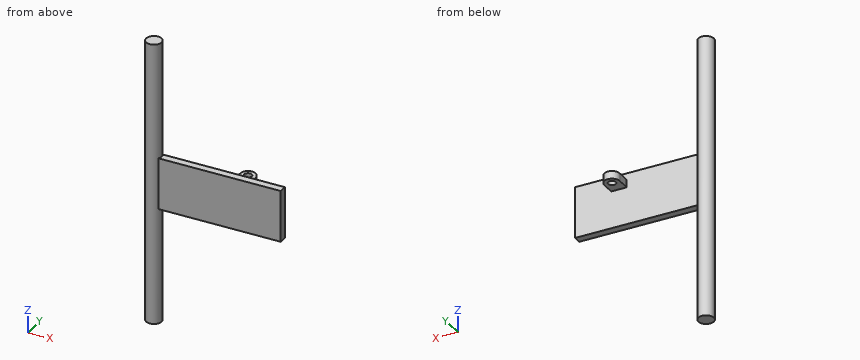
```python
from build123d import *

# Parameters (mm, degrees)
SKETCH1_R           = 3
BOSS_EXTRUDE1_DEPTH = 55
SKETCH2_W           = 50
SKETCH2_H           = 3
BOSS_EXTRUDE2_DEPTH = 10
SKETCH3_R           = 3
SKETCH3_R_2         = 1.5
BOSS_EXTRUDE3_DEPTH = 3


with BuildPart() as part:
    # Sketch1 → Boss-Extrude1 (new, symmetric)
    with BuildSketch(Plane.XY):
        Circle(SKETCH1_R)
    extrude(amount=BOSS_EXTRUDE1_DEPTH, both=True)

    # Sketch2 → Boss-Extrude2 (add, symmetric)
    with BuildSketch(Plane.XY):
        with Locations((25, 0)):
            Rectangle(SKETCH2_W, SKETCH2_H)
    extrude(amount=BOSS_EXTRUDE2_DEPTH, both=True)

    # Sketch3 → Boss-Extrude3 (add)
    # profile 1 of 2: a face of its own
    with BuildSketch(Plane.XY.offset(7.5)):
        with Locations((33, 6.5)):
            Circle(SKETCH3_R)
        with Locations((33, 6.5)):
            Circle(SKETCH3_R_2, mode=Mode.SUBTRACT)
    # profile 2 of 2: a face of its own
    with BuildSketch(Plane.XY.offset(7.5)):
        with BuildLine():
            ThreePointArc((36, 6.5), (33, 3.5), (30, 6.5))
            Line((30, 6.5), (30, 1.5))
            Line((30, 1.5), (36, 1.5))
            Line((36, 1.5), (36, 6.5))
        make_face()
    extrude(amount=-BOSS_EXTRUDE3_DEPTH)


solid = part.part
```
Model file for the job. Use its own axes, mm. Coordinates: 2 decimals unless noted, no trailing zeros. Write each loop counter-clockwise with the first axis right and the second up, starting at its lowest first coordinate (ties: lowest second). Pieces come first, ordered by that corner, then holes. Notation, with made-up numbers: (34, -4) - (46, -4) arc R28 ccw to (46, 25) - close; hole circle Ø11 at (-28.5, 58.25). An arc over 180 degrees is marked (long way). Use a Markdown table: item, result. Add a question column.
Item 1: Drill centre lines: line 1 along Y through (x, z) = (33, 5.45); line 2 along Z through (x, y) = (41, -1); line 3 along Y through (x, z) = (0, 22). Where is each one in solid material? Low to high.
Item 2: Band-saw the part on C-C, the plane z = -19. Write the cut outline in (x, y), and give its area (3 significant figures).
Item 3: Drop flat-ended pins along their axis: pin 1 (3 mm diameter, centred on x = 34, y = 7.5, fed in from +Z); pin 2 (1.5 mm diameter, centred on x = 23, y = 0, fed in from -Z); pin 3 (10 mm diameter, centred on x = 17, z = 2.5, fed in from -Y). Give the stop position or say it passes through.
Item 4: Band-saw the part on D-D, the plane x = 0. Write the cut outline in (y, z).
Item 5: Band-saw the part on B-B, the plane y = 0. Write the cut outline in (x, z), and give its area (3 significant figures).
Item 6: Band-saw the part on A-A, the plane x = 33. Write the cut outline in (y, z), and give its area (3 significant figures).
A:
| question | item | result |
|---|---|---|
| 1 | line 1 | y = -1.5 to 5, 8 to 9.5 |
| 1 | line 2 | z = -10 to 10 |
| 1 | line 3 | y = -3 to 3 |
| 2 | outline | circle Ø6 at (0, 0) |
| 2 | area | 28.3 mm² |
| 3 | pin 1 | stops at z = 7.5 |
| 3 | pin 2 | stops at z = -10 |
| 3 | pin 3 | stops at y = -1.5 |
| 4 | outline | (-3, -55) - (3, -55) - (3, 55) - (-3, 55) - close |
| 5 | outline | (-3, -55) - (3, -55) - (3, -10) - (50, -10) - (50, 10) - (3, 10) - (3, 55) - (-3, 55) - close |
| 5 | area | 1,600 mm² |
| 6 | outline | (-1.5, -10) - (1.5, -10) - (1.5, 4.5) - (5, 4.5) - (5, 7.5) - (1.5, 7.5) - (1.5, 10) - (-1.5, 10) - close; (8, 4.5) - (9.5, 4.5) - (9.5, 7.5) - (8, 7.5) - close |
| 6 | area | 75.0 mm² |
